Print and shaded views of the part. All mm, measured from the part's lowest x, y and z. Round coordinates to 2 decimals unless told otherwise and drop trailing zeros. Loops run counter-clockwise (first coordinate to the right, second up) from the corner with the lowest first, then second, coordinate; pieces in that order, holes last. Notation, with made-up numbers: (-30, 54) -> (-17, 54) arc R34 ccw to (-17, 86) -> close; hole circle Ø6 at (22.25, 31.25). An arc over 180 degrees is marked (long way). Use a Markdown table: item, result.
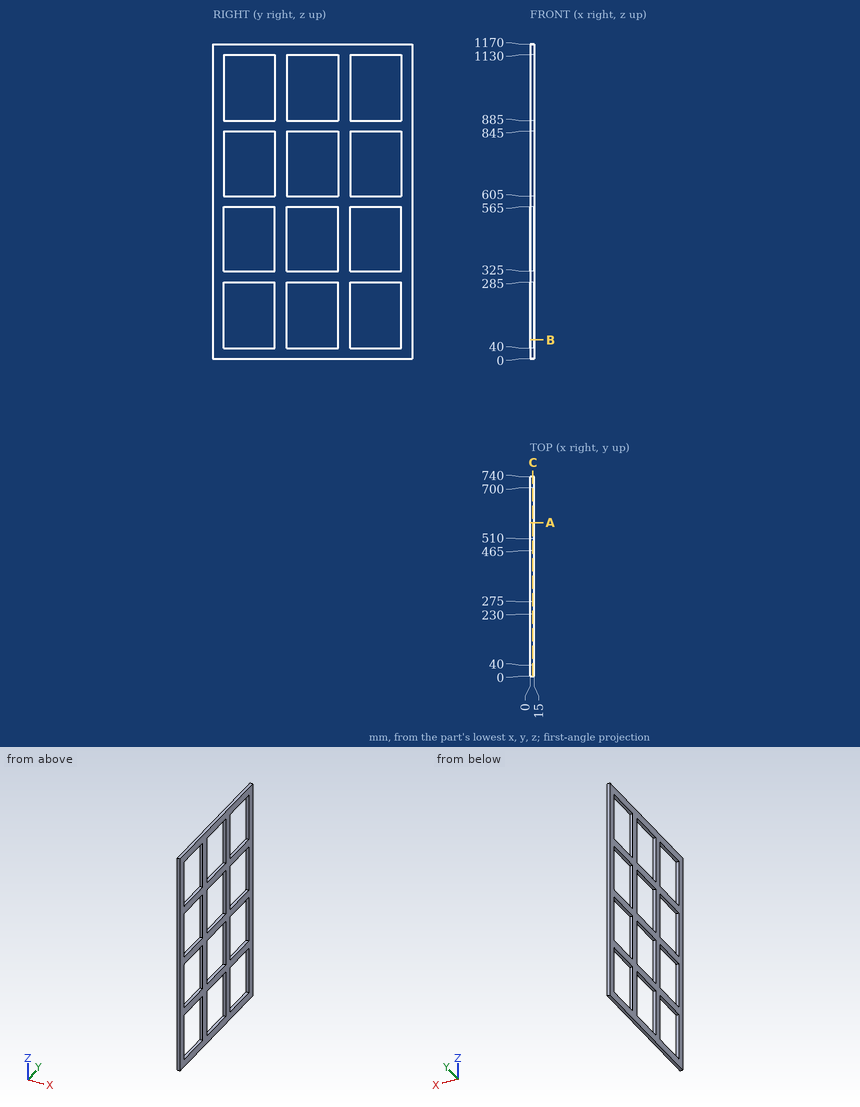
Q1. Band-saw the part on A-A, the plane y = 570. Give the cut face in (x, z), plus the area to 3 significant figures.
Results list:
| item | result |
|---|---|
| outline | (0, 0) -> (15, 0) -> (15, 40) -> (0, 40) -> close; (0, 285) -> (15, 285) -> (15, 325) -> (0, 325) -> close; (0, 565) -> (15, 565) -> (15, 605) -> (0, 605) -> close; (0, 845) -> (15, 845) -> (15, 885) -> (0, 885) -> close; (0, 1130) -> (15, 1130) -> (15, 1170) -> (0, 1170) -> close |
| area | 3,000 mm² |
Q2. Band-saw the part on B-B, the plane z = 70.5. Give the cut face in (x, y), plus the area to 3 significant figures.
Results list:
| item | result |
|---|---|
| outline | (0, 0) -> (15, 0) -> (15, 40) -> (0, 40) -> close; (0, 230) -> (15, 230) -> (15, 275) -> (0, 275) -> close; (0, 465) -> (15, 465) -> (15, 510) -> (0, 510) -> close; (0, 700) -> (15, 700) -> (15, 740) -> (0, 740) -> close |
| area | 2,550 mm² |
Q3. Drill centre lines: L1, parallel to Z at x = 2.25, y = 329; L2, parallel to Y at x = 7, z = 704. Where is each one in solid material? Low to high. Write a range as from..to.
Results list:
| item | result |
|---|---|
| L1 | z = 0..40, 285..325, 565..605, 845..885, 1130..1170 |
| L2 | y = 0..40, 230..275, 465..510, 700..740 |
Q4. Band-saw the part on C-C, the plane x = 10.5. Give the number of separate pieces and of enclosed holes in the cut face, plus the area to 3 significant figures.
Results list:
| item | result |
|---|---|
| separate pieces | 1 |
| enclosed holes | 12 |
| area | 313,000 mm² |
